Read the model definition and answer for the solid it produces. Units are mm, in the model's axes. Round coordinates to 2 decimals unless told otherwise and drop trailing zeros. Loops run counter-clockwise (first coordinate to the right, second up) from the corner with the lowest first, then second, coordinate; pieces in that order, holes last. Notation, with made-up numbers: M 64,74 L 94,74 A27 ccw 94,111 Z; hole C -25.75,87.25 d1. An arc over 180 degrees is marked long. Answer as CSV lines item,"result".
```python
from build123d import *

# Parameters (mm, degrees)
SKETCH1_R           = 50
BOSS_EXTRUDE1_DEPTH = 10
SKETCH2_R           = 5
CUT_EXTRUDE1_DEPTH  = 10
CIRPATTERN1_COUNT   = 3
SKETCH3_R           = 16
CUT_EXTRUDE2_DEPTH  = 10


with BuildPart() as part:
    # Sketch1 → Boss-Extrude1 (new body)
    with BuildSketch(Plane.XY):
        Circle(SKETCH1_R)
    extrude(amount=BOSS_EXTRUDE1_DEPTH)

    # Sketch2 → Cut-Extrude1 (cut)
    with BuildSketch(Plane.XY.offset(10)):
        with Locations((0, 35)):
            Circle(SKETCH2_R)
    cut_extrude1 = extrude(amount=-CUT_EXTRUDE1_DEPTH, mode=Mode.SUBTRACT)

    # CirPattern1: Cut-Extrude1 ×3 about axis
    cirpattern1_axis = Axis((0, 0, 0), (0, 0, 1))
    for i in range(1, CIRPATTERN1_COUNT):
        add(cut_extrude1.rotate(cirpattern1_axis, i * 360 / CIRPATTERN1_COUNT), mode=Mode.SUBTRACT)

    # Sketch3 → Cut-Extrude2 (cut)
    with BuildSketch(Plane.XY.offset(10)):
        Circle(SKETCH3_R)
    extrude(amount=-CUT_EXTRUDE2_DEPTH, mode=Mode.SUBTRACT)


solid = part.part
```
1) Find section A-A, the plane x = 0. Give the vertices of the cut face in (y, z).
Evaluation:
outline,"M -50,0 L -16,0 L -16,10 L -50,10 Z; M 16,0 L 30,0 L 30,10 L 16,10 Z; M 40,0 L 50,0 L 50,10 L 40,10 Z"
2) Find section D-D, the plane y = -19.5. Give the vertices of the cut face in (x, z).
Evaluation:
outline,"M -46.04,0 L -34.89,0 L -34.89,10 L -46.04,10 Z; M -25.73,0 L 25.73,0 L 25.73,10 L -25.73,10 Z; M 34.89,0 L 46.04,0 L 46.04,10 L 34.89,10 Z"
3) Straight lines are drawn through the part: line 1 (Y direction, x = 0, z = 8); line 2 (X direction, y = -16.5, z = 0.75); line 3 (Y direction, x = 4, z = 9). For each, find the intervals that lie inside material, in ascending order.
Evaluation:
line 1,"y = -50 to -16, 16 to 30, 40 to 50"
line 2,"x = -47.2 to -35.21, -25.41 to 25.41, 35.21 to 47.2"
line 3,"y = -49.84 to -15.49, 15.49 to 32, 38 to 49.84"
4) Determine the mould class of faces 1 (the flat face through (-12, 12, 0)), 2 (the cylindrical face through (47.69, 15.02, 4.93)), 3 (the cylindrical face through (3, 39, 5)) for opening direction X: released by +X, released by -X, zero draft, split by the parting line, or undercut.
Evaluation:
face 1,"zero draft"
face 2,"split by the parting line"
face 3,"undercut"
5) Each of these flat-tipped pins is pushed along its axis until it touches: P1, Ø1.5, axis at x = -3, y = -27.5, coming from the -Z side; P2, Ø5, axis at y = 11, z = 8.5, coming from the +X side; P3, Ø6, axis at x = 10, z = 3, coming from the +Y side; P4, Ø4, axis at y = 24.5, z = 5, coming from the -X side. Where does it stop, or does it pass through?
Evaluation:
P1,"stops at z = 0"
P2,"stops at x = 49.27"
P3,"stops at y = 49.51"
P4,"stops at x = -44.65"
6) Find section B-B, the plane y = 4.5. Give the vertices of the cut face in (x, z).
Evaluation:
outline,"M -49.8,0 L -15.35,0 L -15.35,10 L -49.8,10 Z; M 15.35,0 L 49.8,0 L 49.8,10 L 15.35,10 Z"
7) Find section C-C, the plane x = 30.5. Give the vertices of the cut face in (y, z), then the cut area to 3 significant figures.
Evaluation:
outline,"M -39.62,0 L -22.5,0 L -22.5,10 L -39.62,10 Z; M -12.5,0 L 39.62,0 L 39.62,10 L -12.5,10 Z"
area,"692 mm^2"
